```python
from build123d import *

# Parameters (mm, degrees)
SKETCH_1_W      = 50
SKETCH_1_H      = 50
SKETCH_1_W_2    = 44
SKETCH_1_H_2    = 44
EXTRUDE_2_DEPTH = 280


with BuildPart() as part:
    # 草图1 → 凸台-拉伸2 (new body)
    with BuildSketch(Plane.XY):
        with Locations((25, 25)):
            Rectangle(SKETCH_1_W, SKETCH_1_H)
        with Locations((25, 25)):
            Rectangle(SKETCH_1_W_2, SKETCH_1_H_2, mode=Mode.SUBTRACT)
    extrude(amount=EXTRUDE_2_DEPTH)


solid = part.part
```
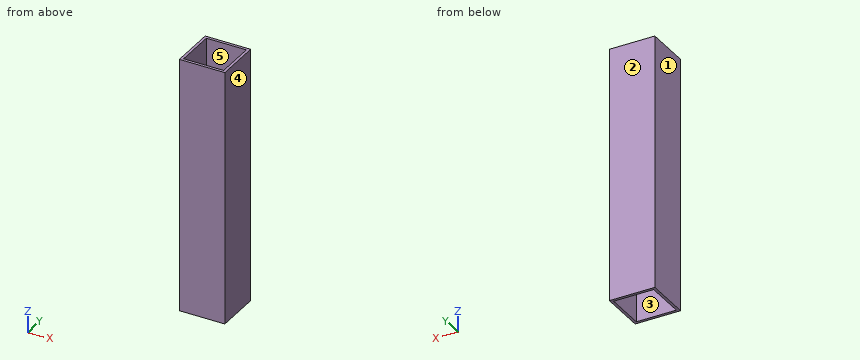
Could you check a few things on this model? Use its own coordinates, in mm. Face numbers are marked on the shaded views. A direction names the side the tool comes from. Coordinates: 2 decimals unless noted, no trailing zeros. Write each loop counter-clockwise with the first axis right and the second up, starting at its lowest first coordinate (ties: lowest second). Pieces come first, ordered by that corner, then holes. Notation, with made-up numbers: (73.5, -33) -> (124.5, -33) arc R28 cw to (124.5, -9) -> close; hole circle Ø9 at (-31, 68.5). An arc over 180 degrees is marked (long way). Write item = value, one per line. Start each with the question number.
(1) I need wall thicknesses on line 1 (Y direction, x = 32, z = 183). Which ranges of the line are inside material? Lowest first, please. Write a range as [from, to].
(2) Will this pin go through, and if not, where does the flat tip stop? pin 1 (5 mm diameter, centred on y = 11, z = 56.5, fed in from -X).
(3) We'd pull the mould along X, two halves only. Please class the marked faces 1, 2 and 3: released by +X, released by -X, zero draft, split by the parting line, or undercut.
(4) I want a section at A-A (z = 30). Please give me the cut outline in (x, y).
(5) Which directions (+Z, -Z, +X, -X, +Y, -Y) give clear straight access to the entire face, cutting with the end or side of a thin tool? Please do the marked faces 4 and 5.
(6) I want a section at B-B (y = 34). Please give me the cut outline in (x, z).
Result set:
q1.line_1 = [0, 3], [47, 50]
q2.pin_1 = 0
q3.face_1 = released by -X
q3.face_2 = zero draft
q3.face_3 = undercut
q4.outline = (0, 0) -> (50, 0) -> (50, 50) -> (0, 50) -> close; hole (3, 3) -> (47, 3) -> (47, 47) -> (3, 47) -> close
q5.face_4 = +Z, -Z, +X, +Y, -Y
q5.face_5 = +Z, -Z
q6.outline = (0, 0) -> (3, 0) -> (3, 280) -> (0, 280) -> close; (47, 0) -> (50, 0) -> (50, 280) -> (47, 280) -> close
